The model under review builds one solid part; all positions refer to its coordinate system, in mm. Face numbers are marked on the shaded views. A direction names the side the tool comes from. Coordinates: 2 decimals unless noted, no trailing zeros. Order: outer loops, then holes, each group sorted by start corner. A loop starts at its lowest first (then second) coordinate and runs counter-clockwise, first axis right, second up. Notation, with made-up numbers: M 58,18 L 72,18 A13 cw 72,33 Z; hole C -39.5,18 d1. An arc over 180 degrees is marked long. Write each question's results on one line, items separated by ' | '.
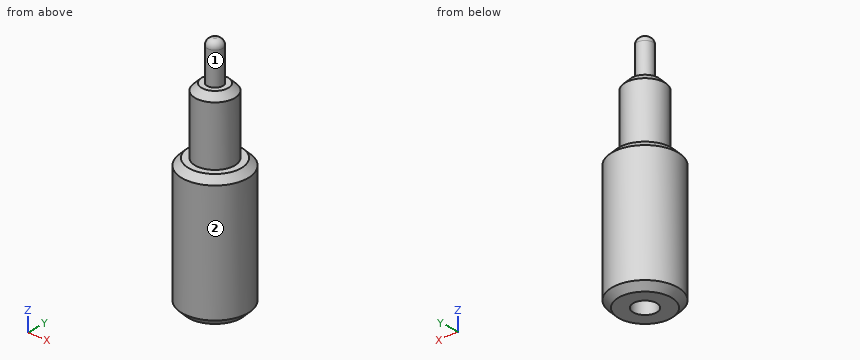
from build123d import *

# Parameters (mm, degrees)
SKETCH1_R           = 2.5
BOSS_EXTRUDE1_DEPTH = 10
SKETCH2_R           = 1.5
BOSS_EXTRUDE2_DEPTH = 5
SKETCH3_R           = 0.6
BOSS_EXTRUDE3_DEPTH = 3
FILLET1_R           = 0.5
SKETCH4_R           = 0.892356389
CUT_EXTRUDE1_DEPTH  = 13
CHAMFER1_SIZE       = 0.5


with BuildPart() as part:
    # Sketch1 → Boss-Extrude1 (new body)
    with BuildSketch(Plane.XY):
        Circle(SKETCH1_R)
    extrude(amount=BOSS_EXTRUDE1_DEPTH)

    # Sketch2 → Boss-Extrude2 (add)
    with BuildSketch(Plane.XY.offset(10)):
        Circle(SKETCH2_R)
    extrude(amount=BOSS_EXTRUDE2_DEPTH)

    # Sketch3 → Boss-Extrude3 (add)
    with BuildSketch(Plane.XY.offset(15)):
        Circle(SKETCH3_R)
    extrude(amount=BOSS_EXTRUDE3_DEPTH)

    # Fillet1
    fillet1_edges = [part.edges().sort_by_distance(p)[0] for p in [
        (-0.6, 0, 18),
    ]]
    fillet(fillet1_edges, radius=FILLET1_R)

    # Sketch4 → Cut-Extrude1 (cut)
    with BuildSketch(Plane(origin=(0, 0, 0), x_dir=(-1, 0, 0), z_dir=(0, 0, -1))):
        Circle(SKETCH4_R)
    extrude(amount=-CUT_EXTRUDE1_DEPTH, mode=Mode.SUBTRACT)

    # Chamfer1
    chamfer1_edges = [part.edges().sort_by_distance(p)[0] for p in [
        (-2.5, 0, 0),
        (-2.5, 0, 10),
        (-1.5, 0, 15),
    ]]
    chamfer(chamfer1_edges, length=CHAMFER1_SIZE)


solid = part.part
1) For pin 1 (1 mm diameter, centred on x = 0.5, z = 15, fed in from -Y); pin 2 (1.5 mm diameter, centred on y = 0, z = 15, fed in from -X); pin 3 (0.5 mm diameter, centred on x = -0.5, y = 0, fed in from -Z), all flat-tipped, find the tip position at first contact; note any pin that passes through.
Solutions:
pin 1: y = -1.44 | pin 2: x = -1.5 | pin 3: z = 13
2) To check wall thickness, follow line 1 along Y through (x, z) = (0, 6.75); line 2 along Z through (x, y) = (0.2, 1.7); line 3 along Y through (x, z) = (0.5, 3.75). State the ranges of each line that lie inside material, in increasing order.
Solutions:
line 1: -2.5 to -0.89, 0.89 to 2.5 | line 2: 0 to 10 | line 3: -2.45 to -0.74, 0.74 to 2.45
3) Take a section at A-A on z = 13.5. State the section outline as (x, y) points.
Solutions:
outline: C 0,0 d3
4) For the marked faces 1 and 2, list the 3-axis set-ups (+Z, -Z, +X, -X, +Y, -Y) from which the entire face can be reached by the end or side of a thin tool; tool diameter is ignored.
Solutions:
face 1: +Z | face 2: +Z, -Z
